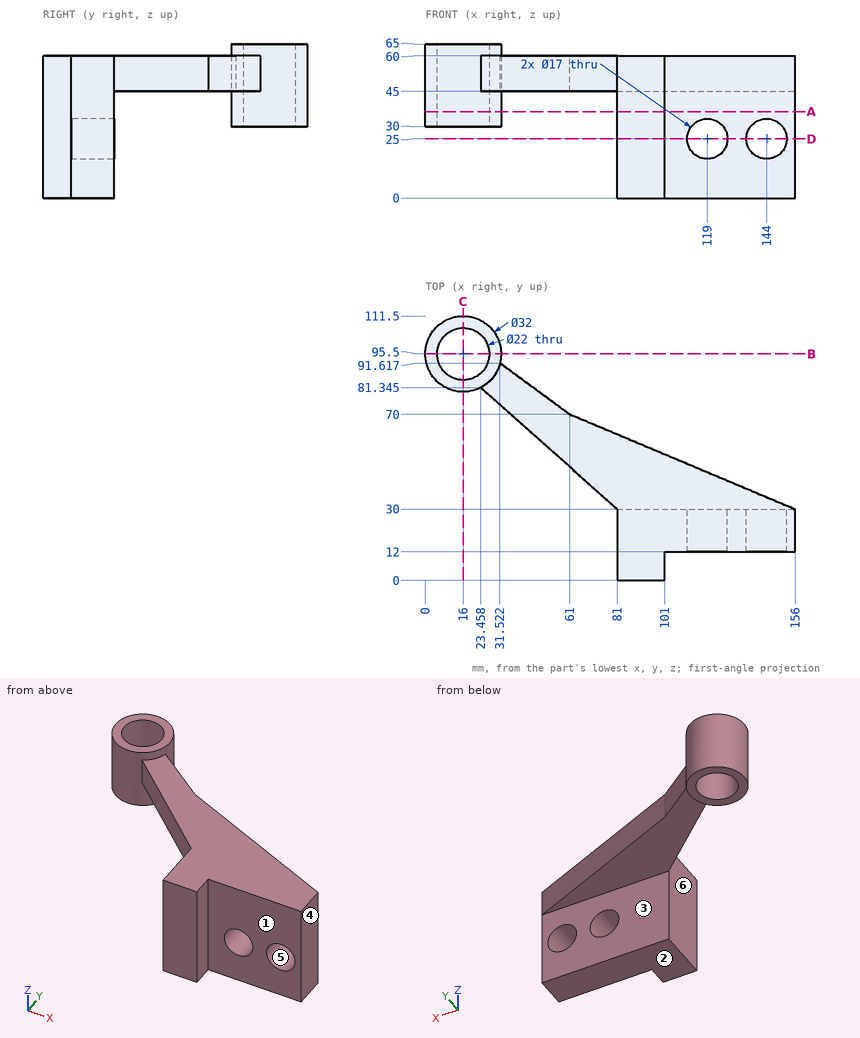
Design review of the part shown in the three views and the two pictorial views. Dimensions are in mm from the part's minimum x, y and z. A direction names the side the tool comes from. Round coordinates to 2 decimals unless told otherwise and drop trailing zeros. Loops run counter-clockwise (first coordinate to the right, second up) from the corner with the lowest first, then second, coordinate; pieces in that order, holes last. Notation, with made-up numbers: M 52,6 L 77,6 A15 ccw 77,13 Z; hole C 68.5,40 d7. An arc over 180 degrees is marked long. Answer as a JSON object with one key per item and string values.
Item 1: We need section A-A on z = 36.5. Give the boundary of the cut face in (x, y), and give its area (3 significant figures).
Answer sheet:
{"outline": "C 16,95.5 d32; M 81,0 L 101,0 L 101,12 L 156,12 L 156,30 L 81,30 Z; hole C 16,95.5 d22", "area": "2,010 mm^2"}
Item 2: We need section C-C on x = 16. Give the boundary of the cut face in (y, z), and give its area (3 significant figures).
Answer sheet:
{"outline": "M 79.5,30 L 84.5,30 L 84.5,65 L 79.5,65 Z; M 106.5,30 L 111.5,30 L 111.5,65 L 106.5,65 Z", "area": "350 mm^2"}
Item 3: The part is to be moulded in two halves that separate along X. For the marked faces 3, 4, 5 and 6, say which applies: pulls with the +X half, pulls with the -X half, needs draft (parallel to the pull), parting line crosses it, or undercut.
Answer sheet:
{"face 3": "needs draft", "face 4": "pulls with the +X half", "face 5": "undercut", "face 6": "pulls with the -X half"}
Item 4: Machinability: for the marked faces 1 and 2, which of the approach directions +Z, -Z, +X, -X, +Y, -Y give a long, thin tool a straight path to every point of the face, cutting with its end or side? Answer none if there is none.
Answer sheet:
{"face 1": "+Z, -Z, +X, -Y", "face 2": "-Z, +X, -X, +Y, -Y"}
Item 5: We need section B-B on y = 95.5. Give the boundary of the cut face in (x, z), and give its area (3 significant figures).
Answer sheet:
{"outline": "M 0,30 L 5,30 L 5,65 L 0,65 Z; M 27,30 L 32,30 L 32,65 L 27,65 Z", "area": "350 mm^2"}
Item 6: Wall thickness on L1, parallel to X at y = 25, z = 25; L2, parallel to Y at x = 16, z = 50; L3, parallel to Z at x = 92.5, y = 28: over which ranges is each line inside the solid? List them lowest first. Write a range as from..to.
Answer sheet:
{"L1": "x = 81..110.5, 127.5..135.5, 152.5..156", "L2": "y = 79.5..84.5, 106.5..111.5", "L3": "z = 0..60"}
Item 7: We need section D-D on z = 25. Give the boundary of the cut face in (x, y).
Answer sheet:
{"outline": "M 81,0 L 101,0 L 101,12 L 110.5,12 L 110.5,30 L 81,30 Z; M 127.5,12 L 135.5,12 L 135.5,30 L 127.5,30 Z; M 152.5,12 L 156,12 L 156,30 L 152.5,30 Z"}
Item 8: Clearance check with flat-ended pins moving along their axes: P1, Ø10, axis at x = 144, z = 25, coming from the +Y side; P2, Ø5, axis at y = 12.5, z = 57.5, coming from the -X side; P3, Ø3, axis at x = 97, y = 54.5, coming from the -Z side; P4, Ø12, axis at x = 123.5, z = 24.5, coming from the +Y side. State where each tip first meets the part, or that it passes through.
Answer sheet:
{"P1": "passes through", "P2": "stops at x = 81", "P3": "stops at z = 45", "P4": "stops at y = 30"}
